Here's how the part is built. I have some questions about the finished solid (model axes, mm). Face numbers are marked on the shaded views. A direction names the side the tool comes from. Round coordinates to 2 decimals unless told otherwise and drop trailing zeros. Write each loop counter-clockwise with the first axis right and the second up, starting at its lowest first coordinate (ties: lowest second). Pieces come first, ordered by that corner, then holes. Notation, with made-up numbers: (35.25, 82.25) - (69.25, 82.25) arc R15 ccw to (69.25, 110.25) - close; hole circle Ø10 at (-27.5, 13.5). An arc over 180 degrees is marked (long way). One line per question, with ' | ' between items. Start each with the question number.
(1) Imagine slicing it at C-C (z = -2.6). Write out the boundary of the cut face in (x, y), plus the area to 3 significant figures.
(2) Will these pins go through, and if not, where does the flat tip stop? pin 1 (4 mm diameter, centred on y = 8.5, z = -4, fed in from -X); pin 2 (2 mm diameter, centred on x = -3.5, z = -0.5, fed in from +Y); pin 3 (3.5 mm diameter, centred on x = -2.25, z = 2.6, fed in from +Y); pin 4 (2 mm diameter, centred on y = 9.3, z = 2, fed in from +X).
(3) Imagine slicing it at B-B (x = -2.25). Write out the boundary of the cut face in (y, z), plus the area to 3 significant figures.
(4) Imagine slicing it at A-A (y = 9.3). Write out the boundary of the cut face in (x, z), plus the area to 4 significant figures.
(5) For the marked faces 1 and 2, which set-ups out of +Z, -Z, +X, -X, +Y, -Y let a thin tool reach every point of the face, with its end or its side?
(6) If I drill on L1, parallel to Y at x = 4.45, z = 2; L2, parallel to Z at x = -3.5, y = 1.5; L3, parallel to Y at x = -2, z = 4.75, over which ranges is the centre line in solid material (lowest first)?
(7) Thinking about a two-plate mould opening in X: for the marked faces 3, 4 and 5, which applies, pulls with the +X half, pulls with the -X half, needs draft (parallel to the pull), parting line crosses it, or undercut?
(8) Imagine slicing it at D-D (y = 1). Write out the boundary of the cut face in (x, z), plus the area to 3 significant figures.
from build123d import *

# Parameters (mm, degrees)
SKETCH1_W             = 11
SKETCH1_H             = 11
BOSS_EXTRUDE1_DEPTH   = 3
SKETCH2_W             = 4.5
SKETCH2_H             = 11
BOSS_EXTRUDE2_DEPTH   = 9.3
M3_TAPPED_HOLE1_D     = 2.5
M3_TAPPED_HOLE1_DEPTH = 8.5
M3_TAPPED_HOLE1_TIP   = 0.751075774
SKETCH5_R             = 1.6
CUT_EXTRUDE1_DEPTH    = 13.123943253
CHAMFER1_SIZE         = 0.5


with BuildPart() as part:
    # Sketch1 → Boss-Extrude1 (new body)
    with BuildSketch(Plane(origin=(0, 0, 0), x_dir=(1, 0, 0), z_dir=(0, 1, 0))):
        Rectangle(SKETCH1_W, SKETCH1_H)
    extrude(amount=BOSS_EXTRUDE1_DEPTH)

    # Sketch2 → Boss-Extrude2 (add)
    with BuildSketch(Plane(origin=(0, 3, 0), x_dir=(1, 0, 0), z_dir=(0, 1, 0))):
        with Locations((3.25, 0)):
            Rectangle(SKETCH2_W, SKETCH2_H)
    extrude(amount=BOSS_EXTRUDE2_DEPTH)

    # M3 Tapped Hole1
    with Locations(Plane.ZY.offset(-1)):
        with Locations((2, 9.3)):
            Hole(M3_TAPPED_HOLE1_D / 2, depth=M3_TAPPED_HOLE1_DEPTH)
            with Locations((0, 0, -(M3_TAPPED_HOLE1_DEPTH + M3_TAPPED_HOLE1_TIP / 2))):  # 118° drill point
                Cone(0, M3_TAPPED_HOLE1_D / 2, M3_TAPPED_HOLE1_TIP, mode=Mode.SUBTRACT)

    # Sketch5 → Cut-Extrude1 (cut, through all)
    with BuildSketch(Plane(origin=(0, 3, 0), x_dir=(1, 0, 0), z_dir=(0, 1, 0))):
        with Locations(Location((-2.25, 2.6, 0), (0, 0, 270))):
            Circle(SKETCH5_R)
        with Locations(Location((-2.25, -2.6, 0), (0, 0, 270))):
            Circle(SKETCH5_R)
    extrude(amount=-CUT_EXTRUDE1_DEPTH, mode=Mode.SUBTRACT)

    # Chamfer1
    chamfer1_edges = [part.edges().sort_by_distance(p)[0] for p in [
        (-2.25, 3, -4.2),
        (-2.25, 3, 1),
    ]]
    chamfer(chamfer1_edges, length=CHAMFER1_SIZE)


solid = part.part
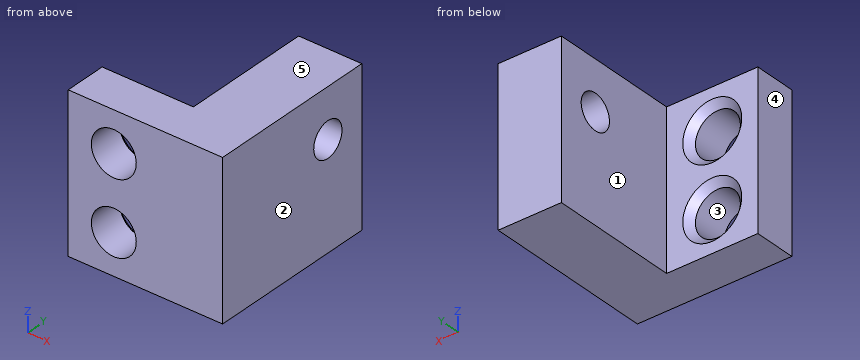
Check sheet entries:
1) outline: (-5.5, 0) - (-3.85, 0) - (-3.85, 2.5) - (-4.35, 3) - (-5.5, 3) - close; (-0.65, 0) - (5.5, 0) - (5.5, 12.3) - (1, 12.3) - (1, 3) - (-0.15, 3) - (-0.65, 2.5) - close | area: 65.0 mm^2
2) pin 1: x = 1 | pin 2: y = 3 | pin 3: y = 2.65 | pin 4: through
3) outline: (0, -5.5) - (3, -5.5) - (3, -4.7) - (2.5, -4.2) - (0, -4.2) - close; (0, -1) - (2.5, -1) - (3, -0.5) - (3, 0.5) - (2.5, 1) - (0, 1) - close; (0, 4.2) - (2.5, 4.2) - (3, 4.7) - (3, 5.5) - (0, 5.5) - close | area: 13.3 mm^2
4) outline: (1, -5.5) - (5.5, -5.5) - (5.5, 0.75) - (1, 0.75) - close; (1, 3.25) - (5.5, 3.25) - (5.5, 5.5) - (1, 5.5) - close | area: 38.25 mm^2
5) face 1: +Z, -Z, -X, +Y | face 2: +Z, -Z, +X, +Y, -Y
6) L1: 0 to 8.05, 10.55 to 12.3 | L2: -5.5 to -3.6, -1.6 to 1.6, 3.6 to 5.5 | L3: 0 to 3
7) face 3: undercut | face 4: pulls with the -X half | face 5: needs draft
8) outline: (-5.5, -5.5) - (5.5, -5.5) - (5.5, 5.5) - (-5.5, 5.5) - close; hole circle Ø3.2 at (-2.25, -2.6); hole circle Ø3.2 at (-2.25, 2.6) | area: 105 mm^2
